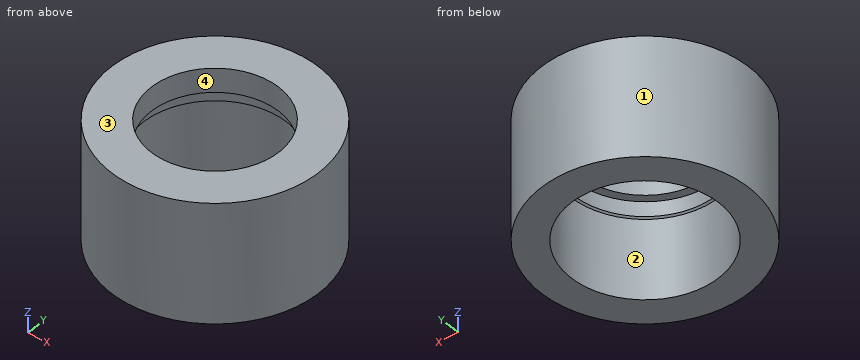
from build123d import *


with BuildPart() as part:
    # Sketch1 → Revolve1 (revolve)
    with BuildSketch(Plane.XZ, mode=Mode.PRIVATE) as revolve1_sk:
        Polygon((9.25, 0), (13, 0), (13, 15), (8, 15), (8, 12), (9, 12), (9, 10.150215155), (9.25, 10), align=None)
    revolve(revolve1_sk.sketch.rotate(Axis((0, 0, 15), (0, 0, -1)), 180), axis=Axis((0, 0, 15), (0, 0, -1)))


solid = part.part
Read the model definition and answer for the solid it produces. Units are mm, in the model's axes. Face numbers are marked on the shaded views. Give positions to 0.01 mm unless a question says otherwise; leave off trailing zeros. Write each loop counter-clockwise with the first axis right and the second up, starting at its lowest first coordinate (ties: lowest second). Pieces come first, ordered by that corner, then holes. Notation, with made-up numbers: (66.25, 87.25) - (71.25, 87.25) arc R35 cw to (71.25, 122.25) - close; hole circle Ø9 at (-16, 27.25). An arc over 180 degrees is marked (long way). Answer in a Markdown table with one row per item. Add a question column.
Item 1: Section C-C, the plane z = 8.5 is taken. Write down the section's boundary in (x, y), and give its area (3 significant figures).
Item 2: Determine the mould class of the marked faces 1, 2, 3 and 4 for opening direction Y: pulls with the +Y half, pulls with the -Y half, needs draft (parallel to the pull), parting line crosses it, or undercut.
Item 3: Section A-A, the plane y = 0 is taken. Write down the section's boundary in (x, z), and give its area (3 significant figures).
Item 4: Find the intervals of material crossed by L1, parallel to Y at x = 0, z = 6.5; L2, parallel to Y at x = -7.5, z = 4, in increasing order.
Item 5: Section D-D, the plane z = 14.25 is taken. Write down the section's boundary in (x, y), and give its area (3 significant figures).
Item 6: Flat-ended cylindrical pins translate along their axes: P1, Ø3, axis at x = -4.5, z = 8, coming from the +Y side; P2, Ø6, axis at x = 8.5, z = 10.5, coming from the +Y side; P3, Ø1, axis at y = -1, z = 9.5, coming from the -X side. Find the tip coordinate at first contact, or state that the pin passes through.
Recorded:
| question | item | result |
|---|---|---|
| 1 | outline | circle Ø26 at (0, 0); hole circle Ø18.5 at (0, 0) |
| 1 | area | 262 mm2 |
| 2 | face 1 | parting line crosses it |
| 2 | face 2 | undercut |
| 2 | face 3 | needs draft |
| 2 | face 4 | undercut |
| 3 | outline | (-13, 0) - (-9.25, 0) - (-9.25, 10) - (-9, 10.15) - (-9, 12) - (-8, 12) - (-8, 15) - (-13, 15) - close; (8, 12) - (9, 12) - (9, 10.15) - (9.25, 10) - (9.25, 0) - (13, 0) - (13, 15) - (8, 15) - close |
| 3 | area | 121 mm2 |
| 4 | L1 | y = -13 to -9.25, 9.25 to 13 |
| 4 | L2 | y = -10.62 to -5.41, 5.41 to 10.62 |
| 5 | outline | circle Ø26 at (0, 0); hole circle Ø16 at (0, 0) |
| 5 | area | 330 mm2 |
| 6 | P1 | stops at y = 12.65 |
| 6 | P2 | stops at y = 11.78 |
| 6 | P3 | stops at x = -12.99 |
